Input: part model. Units: mm. Frame: model coordinates. A direction names the side the tool comes from. Give positions to 0.01 mm unless a question says otherwise; leave off trailing zeros. Loops run counter-clockwise (first coordinate to the right, second up) from the corner with the lowest first, then second, coordinate; pieces in that order, holes last.
from build123d import *

# Parameters (mm, degrees)
SKETCH_1_R          = 1.64
SKETCH_1_R_2        = 1.15
EXTRUDE_1_DEPTH     = 3.1
EXTRUDE_1_2_DEPTH   = 3.1
EXTRUDE_START       = -3.1
EXTRUDE_2_DEPTH     = 3.1
SKETCH_4_W          = 9.63
SKETCH_4_H          = 10
EXTRUDE_3_DEPTH     = 5.6
SKETCH_5_W          = 4.83
SKETCH_5_H          = 5.53
CUT_EXTRUDE_1_DEPTH = 10
SKETCH_6_W          = 4.83
SKETCH_6_H          = 7.53
CUT_EXTRUDE_2_DEPTH = 1.5
SKETCH_7_W          = 2.070948157
SKETCH_7_H          = 7.64
EXTRUDE_4_DEPTH     = 9.63
SKETCH_10_R         = 1.15
CUT_EXTRUDE_3_DEPTH = 22.934678024
SKETCH_11_W         = 3.1
SKETCH_11_H         = 7.64
CUT_EXTRUDE_4_DEPTH = 21.601623722
CUT_EXTRUDE_5_DEPTH = 22.934678024


with BuildPart() as part:
    # Sketch 1 → Extrude 1 (new body)
    with BuildSketch(Plane.XY):
        with Locations(Location((0, 0, 0), (0, 0, 180))):
            Circle(SKETCH_1_R)
        with Locations(Location((0, 0, 0), (0, 0, 180))):
            Circle(SKETCH_1_R_2, mode=Mode.SUBTRACT)
    extrude(amount=EXTRUDE_1_DEPTH)



with BuildPart() as body_2:
    # Sketch 1 → Extrude 1 2 (new body)
    with BuildSketch(Plane.XY):
        with Locations(Location((-6.35, 0, 0), (0, 0, 180))):
            Circle(SKETCH_1_R)
        with Locations(Location((-6.35, 0, 0), (0, 0, 180))):
            Circle(SKETCH_1_R_2, mode=Mode.SUBTRACT)
    extrude(amount=EXTRUDE_1_2_DEPTH)


with BuildPart() as part_1:
    add(part.part)

    add(body_2.part)  # Extrude 2 merges body 2
    # Sketch 2 → Extrude 2 (add)
    with BuildSketch(Plane.XY.offset(3.1).offset(EXTRUDE_START)):
        with BuildLine():
            Line((-7.99, 0), (-7.99, 16))
            Line((-7.99, 16), (1.64, 16))
            Line((1.64, 16), (1.64, 0))
            ThreePointArc((1.64, 0), (0, 1.64), (-1.64, 0))
            Line((-1.64, 0), (-4.71, 0))
            ThreePointArc((-4.71, 0), (-6.35, 1.64), (-7.99, 0))
        make_face()
    extrude(amount=EXTRUDE_2_DEPTH)

    # Sketch 4 → Extrude 3 (add)
    with BuildSketch(Plane.XY.offset(3.1)):
        with Locations((-3.175, 11)):
            Rectangle(SKETCH_4_W, SKETCH_4_H)
    extrude(amount=EXTRUDE_3_DEPTH)

    # Sketch 5 → Cut-Extrude 1 (cut)
    with BuildSketch(Plane.XY.offset(8.7)):
        with Locations((-3.175, 10.85)):
            Rectangle(SKETCH_5_W, SKETCH_5_H)
    extrude(amount=-CUT_EXTRUDE_1_DEPTH, mode=Mode.SUBTRACT)

    # Sketch 6 → Cut-Extrude 2 (cut)
    with BuildSketch(Plane.XY.offset(7.2)):
        with Locations((-3.175, 10.85)):
            Rectangle(SKETCH_6_W, SKETCH_6_H)
    extrude(amount=-CUT_EXTRUDE_2_DEPTH, mode=Mode.SUBTRACT)

    # Sketch 7 → Extrude 4 (add)
    with BuildSketch(Plane.ZY.offset(7.99)):
        with Locations((6.206422236, 2.18)):
            Rectangle(SKETCH_7_W, SKETCH_7_H)
        Polygon((0, 6), (-2, 6), (-2, -1.64), (-4, -1.64), (-4, 6), (-4, 7), (0, 7), align=None)
    extrude(amount=-EXTRUDE_4_DEPTH)

    # Sketch 10 → Cut-Extrude 3 (cut, through all)
    with BuildSketch(Plane(origin=(0, 0, -4), x_dir=(-1, 0, 0), z_dir=(0, 0, -1))):
        Circle(SKETCH_10_R)
        with Locations((6.35, 0)):
            Circle(SKETCH_10_R)
    extrude(amount=-CUT_EXTRUDE_3_DEPTH, mode=Mode.SUBTRACT)

    # Sketch 11 → Cut-Extrude 4 (cut, through all)
    with BuildSketch(Plane(origin=(1.64, 0, 0), x_dir=(0, 0, -1), z_dir=(1, 0, 0))):
        with Locations((-1.55, 2.18)):
            Rectangle(SKETCH_11_W, SKETCH_11_H)
    extrude(amount=-CUT_EXTRUDE_4_DEPTH, mode=Mode.SUBTRACT)

    # Sketch 12 → Cut-Extrude 5 (cut, through all)
    with BuildSketch(Plane(origin=(0, 0, -4), x_dir=(-1, 0, 0), z_dir=(0, 0, -1))):
        with BuildLine():
            Line((4.71, 0), (1.64, 0))
            ThreePointArc((1.64, 0), (1.159655121, -1.159655121), (0, -1.64))
            Line((0, -1.64), (6.35, -1.64))
            ThreePointArc((6.35, -1.64), (5.190344879, -1.159655121), (4.71, 0))
        make_face()
        with BuildLine():
            Line((-1.64, -1.64), (0, -1.64))
            ThreePointArc((0, -1.64), (-1.159655121, -1.159655121), (-1.64, 0))
            Line((-1.64, 0), (-1.64, -1.64))
        make_face()
        with BuildLine():
            ThreePointArc((7.99, 0), (7.509655121, -1.159655121), (6.35, -1.64))
            Line((6.35, -1.64), (7.99, -1.64))
            Line((7.99, -1.64), (7.99, 0))
        make_face()
    extrude(amount=-CUT_EXTRUDE_5_DEPTH, mode=Mode.SUBTRACT)


solid = part_1.part
(1) Ray query, probe 1 along Z at (x, y) = (-7.5, 3.75); probe 2 along Y at (x, z) = (0, -3.2); probe 3 along X at (y, z) = (13.5, 6). Return the intervals inside material, ascending.
Values follow:
probe 1: z = -4 to -2, 5.17 to 7.24
probe 2: y = -1.64 to -1.15, 1.15 to 7
probe 3: x = -7.99 to -5.59, -0.76 to 1.64
(2) Pin query (flat end, axial travel): pin 1 Ø2.5 at (x, y) = (-1, 10.5) entering from -Z; pin 2 Ø1.5 at (x, y) = (-6.5, 0.5) entering from -Z; pin 3 Ø1.5 at (x, z) = (-5, 6) entering from -Y; pin 4 Ø5.5 at (x, z) = (-4, 1.5) entering from -Y. Return the tip coordinate at first contact, or that it passes through.
Values follow:
pin 1: stops at z = 0
pin 2: stops at z = -4
pin 3: stops at y = -1.53
pin 4: stops at y = 6
(3) Mould query, pull axis Z, two halves, no side actions, for faces 1 (the flat face through (-3, 4, -4)), 2 (the flat face through (-3, 7.085, 6)), 3 (the flat face through (-3, 0, 6)). Classes: +Z half, -Z half, draft (parallel to the pull), parting line (faces both ways), or undercut.
Values follow:
face 1: -Z half
face 2: undercut
face 3: draft
(4) Cut plane C-C (z = 4.75). Return the cut outline in (x, y) (3 decimals), and give its area (3 significant figures).
Values follow:
outline: (-7.99, 6) - (1.64, 6) - (1.64, 16) - (-7.99, 16) - close; hole (-5.59, 8.085) - (-0.76, 8.085) - (-0.76, 13.615) - (-5.59, 13.615) - close
area: 69.6 mm2
(5) Cut plane B-B (x = -3.5). Return the cut outline in (y, z) (3 decimals).
Values follow:
outline: (0, -4) - (7, -4) - (7, 0) - (8.085, 0) - (8.085, 5.7) - (7.085, 5.7) - (7.085, 7.2) - (8.085, 7.2) - (8.085, 8.7) - (6, 8.7) - (6, 7.242) - (0, 7.242) - (0, 5.171) - (6, 5.171) - (6, -2) - (0, -2) - close; (13.615, 0) - (16, 0) - (16, 8.7) - (13.615, 8.7) - (13.615, 7.2) - (14.615, 7.2) - (14.615, 5.7) - (13.615, 5.7) - close
(6) Cut plane A-A (y = 1.75). Return the cut outline in (x, z), and give its area (3 significant figures).
Values follow:
outline: (-7.99, -4) - (1.64, -4) - (1.64, -2) - (-7.99, -2) - close; (-7.99, 5.17) - (1.64, 5.17) - (1.64, 7.24) - (-7.99, 7.24) - close
area: 39.2 mm2
(7) Cut plane D-D (y = 9.75). Return the cut outline in (x, z), and give its area (3 significant figures).
Values follow:
outline: (-7.99, 0) - (-5.59, 0) - (-5.59, 8.7) - (-7.99, 8.7) - close; (-0.76, 0) - (1.64, 0) - (1.64, 8.7) - (-0.76, 8.7) - close
area: 41.8 mm2
(8) Reachability of faces 4 (the flat face through (-3, 6, 8)), 5 (the flat face through (-3, 3, -2)), 6 (the flat face through (-3, 7, -2)), 7 (the flat face through (-3.2, 7.6, 7.2)) from +Z, -Z, +X, -X, +Y, -Y: full face, straight path, thin tool, end or side. Return the list, or none.
Values follow:
face 4: +Z, +X, -X, -Y
face 5: +X, -X, -Y
face 6: -Z, +X, -X, +Y
face 7: none
